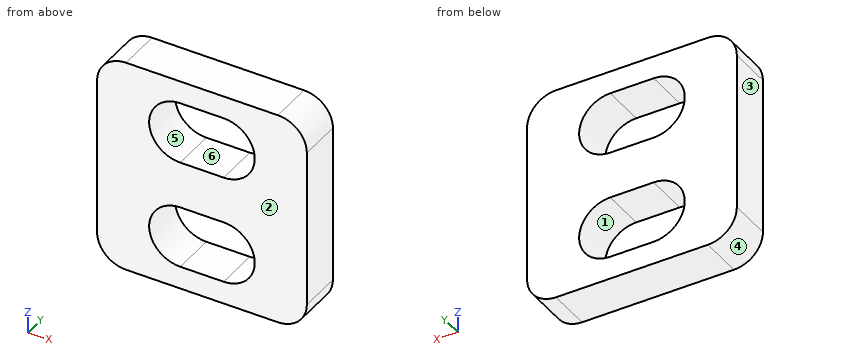
```python
from build123d import *

# Parameters (mm, degrees)
SKETCH_1_W          = 14.5
SKETCH_1_H          = 15
EXTRUDE_1_DEPTH     = 3
CUT_EXTRUDE_1_DEPTH = 10
FILLET_1_R          = 2


with BuildPart() as part:
    # 草图1 → 凸台-拉伸1 (new body)
    with BuildSketch(Plane(origin=(0, 0, 0), x_dir=(1, 0, 0), z_dir=(0, 1, 0))):
        Rectangle(SKETCH_1_W, SKETCH_1_H)
    extrude(amount=EXTRUDE_1_DEPTH)

    # 草图4 → 切除-拉伸1 (cut)
    with BuildSketch(Plane.XZ):
        with BuildLine():
            Line((1.5, -5.922481842), (-1.5, -5.922481842))
            ThreePointArc((-1.5, -5.922481842), (-3.65, -3.772481842), (-1.5, -1.622481842))
            Line((-1.5, -1.622481842), (1.5, -1.622481842))
            ThreePointArc((1.5, -1.622481842), (3.65, -3.772481842), (1.5, -5.922481842))
        make_face()
        with BuildLine():
            Line((1.5, 5.922481842), (-1.5, 5.922481842))
            ThreePointArc((-1.5, 5.922481842), (-3.65, 3.772481842), (-1.5, 1.622481842))
            Line((-1.5, 1.622481842), (1.5, 1.622481842))
            ThreePointArc((1.5, 1.622481842), (3.65, 3.772481842), (1.5, 5.922481842))
        make_face()
    extrude(amount=-CUT_EXTRUDE_1_DEPTH, mode=Mode.SUBTRACT)

    # 圆角1
    fillet_1_edges = [part.edges().sort_by_distance(p)[0] for p in [
        (7.25, 1.5, 7.5),
        (-7.25, 1.5, 7.5),
        (-7.25, 1.5, -7.5),
        (7.25, 1.5, -7.5),
    ]]
    fillet(fillet_1_edges, radius=FILLET_1_R)


solid = part.part
```
Input: part model. Units: mm. Frame: model coordinates. Face numbers are marked on the shaded views. A direction names the side the tool comes from. Round coordinates to 2 decimals unless told otherwise and drop trailing zeros. Loops run counter-clockwise (first coordinate to the right, second up) from the corner with the lowest first, then second, coordinate; pieces in that order, holes last. Notation, with made-up numbers: (44, 11.5) -> (81, 11.5) arc R28 ccw to (81, 44.5) -> close; hole circle Ø7 at (41, 81.25). An arc over 180 degrees is marked (long way). One line per item, written item: value.
(1) Section B-B (y = 2.5). Return the cut outline in (x, z).
Geometry check:
outline: (-7.25, -5.5) arc R2 ccw to (-5.25, -7.5) -> (5.25, -7.5) arc R2 ccw to (7.25, -5.5) -> (7.25, 5.5) arc R2 ccw to (5.25, 7.5) -> (-5.25, 7.5) arc R2 ccw to (-7.25, 5.5) -> close; hole (-1.5, -5.92) -> (1.5, -5.92) arc R2.15 ccw to (1.5, -1.62) -> (-1.5, -1.62) arc R2.15 ccw to start; hole (-1.5, 1.62) -> (1.5, 1.62) arc R2.15 ccw to (1.5, 5.92) -> (-1.5, 5.92) arc R2.15 ccw to start
(2) Section A-A (x = -1.25). Return the cut outline in (y, z).
Geometry check:
outline: (0, -7.5) -> (3, -7.5) -> (3, -5.92) -> (0, -5.92) -> close; (0, -1.62) -> (3, -1.62) -> (3, 1.62) -> (0, 1.62) -> close; (0, 5.92) -> (3, 5.92) -> (3, 7.5) -> (0, 7.5) -> close
(3) Section D-D (z = 2). Return the cut outline in (x, y).
Geometry check:
outline: (-7.25, 0) -> (-2.72, 0) -> (-2.72, 3) -> (-7.25, 3) -> close; (2.72, 0) -> (7.25, 0) -> (7.25, 3) -> (2.72, 3) -> close
(4) Material intervals for line 1 (Z direction, x = 0.75, y = 0.45); line 2 (X direction, y = 1.35, z = -3.75); line 3 (Z direction, x = -2.5, y = 1.9), sorted ascending. Write a range as [from, to].
Geometry check:
line 1: [-7.5, -5.92], [-1.62, 1.62], [5.92, 7.5]
line 2: [-7.25, -3.65], [3.65, 7.25]
line 3: [-7.5, -5.68], [-1.87, 1.87], [5.68, 7.5]
(5) Mould query, pull axis Z, two halves, no side actions, for the marked faces 3, 4, 5 and 6. Classes: pulls with the +Z half, pulls with the -Z half, needs draft (parallel to the pull), parting line crosses it, or undercut.
Geometry check:
face 3: needs draft
face 4: pulls with the -Z half
face 5: undercut
face 6: undercut
(6) Set-up query: the marked faces 1 and 2. Return all of +Z, -Z, +X, -X, +Y, -Y with unobstructed straight access to the full face (end or side cutting, diameter ignored); none if empty.
Geometry check:
face 1: +Y, -Y
face 2: +Z, -Z, +X, -X, -Y
(7) Section C-C (z = 4.5). Return the cut outline in (x, y), plus the area to 3 significant figures.
Geometry check:
outline: (-7.25, 0) -> (-3.52, 0) -> (-3.52, 3) -> (-7.25, 3) -> close; (3.52, 0) -> (7.25, 0) -> (7.25, 3) -> (3.52, 3) -> close
area: 22.4 mm2
